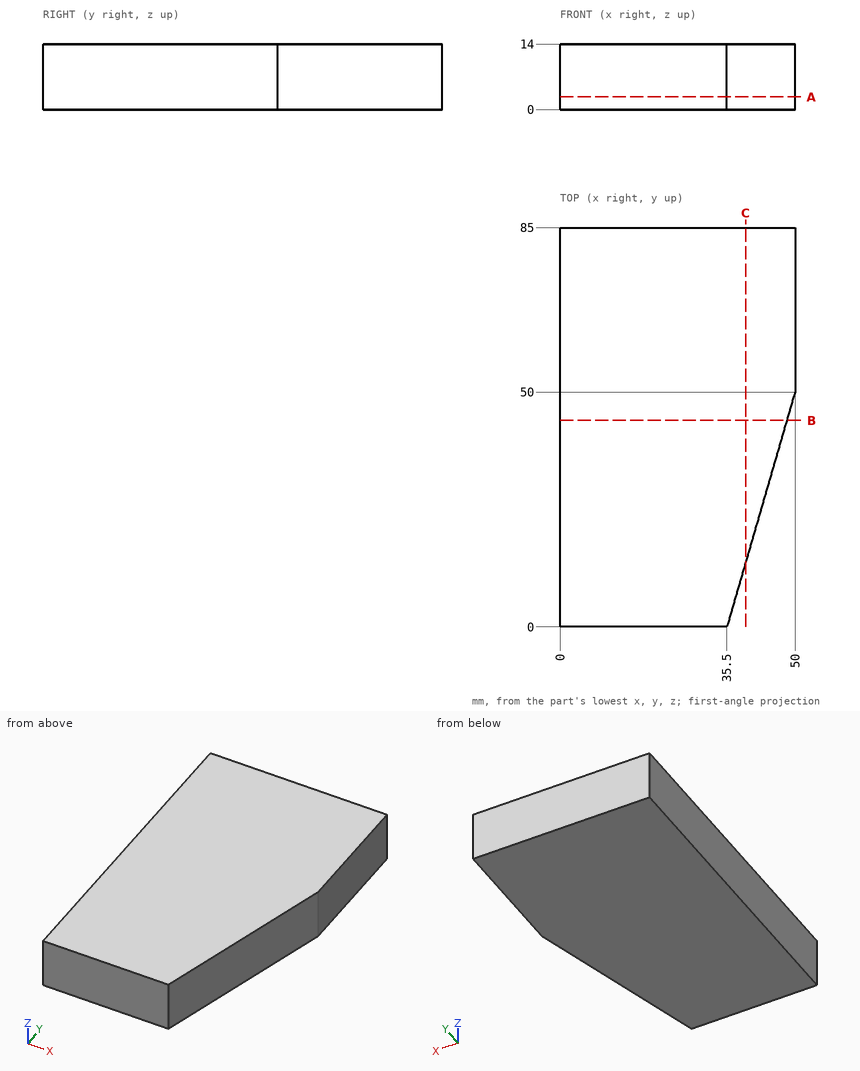
Job drawing, mm, ordinate dimensions from the low corner. One solid piece. Give positions to 0.01 mm unless a question says otherwise; leave off trailing zeros. Order: outer loops, then holes, each group sorted by start corner. A loop starts at its lowest first (then second) coordinate and runs counter-clockwise, first axis right, second up. Notation, with made-up numbers: (66, -7.75) - (97, -7.75) arc R24 ccw to (97, 8.25) - close; hole circle Ø5 at (74.25, -17.5). An arc over 180 degrees is marked (long way). Return JSON: item names as keys, results as strings.
1) Probe line 1 (X direction, y = 17, z = 1); line 2 (X direction, y = 5, z = 11.25). List the from-to ranges inside material, lowest first. Write a range as from..to.
Geometry says:
{"line 1": "0..40.43", "line 2": "0..36.95"}
2) Cut at C-C, the plane x = 39.5. Give the cut face in (y, z).
Geometry says:
{"outline": "(13.79, 0) - (85, 0) - (85, 14) - (13.79, 14) - close"}
3) Cut at A-A, the plane z = 2.75. Give the cut face in (x, y).
Geometry says:
{"outline": "(0, 0) - (35.5, 0) - (50, 50) - (50, 85) - (0, 85) - close"}
4) Cut at B-B, the plane y = 44. Give the cut face in (x, z), plus the area to 3 significant figures.
Geometry says:
{"outline": "(0, 0) - (48.26, 0) - (48.26, 14) - (0, 14) - close", "area": "676 mm²"}
